Read the model definition and answer for the solid it produces. Units are mm, in the model's axes. Face numbers are marked on the shaded views. A direction names the side the tool comes from. Round coordinates to 2 decimals unless told otherwise and drop trailing zeros. Loops run counter-clockwise (first coordinate to the right, second up) from the corner with the lowest first, then second, coordinate; pieces in that order, holes last. Notation, with made-up numbers: M 64,86 L 86,86 A23 ccw 86,94 Z; hole C -1,18 d11. An arc over 180 degrees is marked long. Write each question's results on one line, items separated by ' | '.
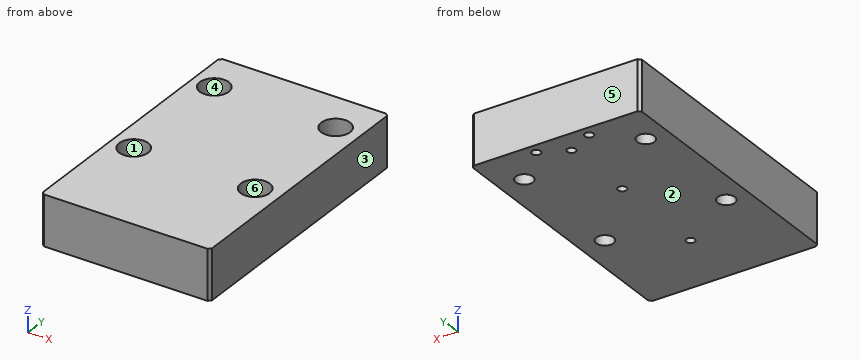
```python
from build123d import *

# Parameters (mm, degrees)
SKETCH_15_W                  = 44
SKETCH_15_H                  = 120
EXTRUDE_1_DEPTH              = 19
HOLE_WIZARD_M4_2_D           = 3.3
HOLE_WIZARD_M4_2_DEPTH       = 11.5
HOLE_WIZARD_M4_2_TIP         = 0.991420021
SKETCH_21_W                  = 44
SKETCH_21_H                  = 18
CUT_EXTRUDE_4_DEPTH          = 19
HOLE_WIZARD_M4_1_D           = 3.3
HOLE_WIZARD_M4_1_DEPTH       = 10.1
HOLE_WIZARD_M4_1_TIP         = 0.991420021
CHAMFER_1_SIZE               = 1
SKETCH_24_W                  = 13.771291576
SKETCH_24_H                  = 102
SKETCH_24_W_2                = 13.032581782
EXTRUDE_2_DEPTH              = 19
HOLE_WIZARD_M6_1_D           = 6.6
HOLE_WIZARD_M6_1_CBORE_D     = 11
HOLE_WIZARD_M6_1_CBORE_DEPTH = 6.4
CHAMFER_2_SIZE               = 1


with BuildPart() as part:
    # 草图15 → 凸台-拉伸1 (new body)
    with BuildSketch(Plane.XY):
        with Locations((3.072247365, -30.72304468)):
            Rectangle(SKETCH_15_W, SKETCH_15_H)
    extrude(amount=EXTRUDE_1_DEPTH)

    # M4 螺纹孔2
    with Locations(Plane(origin=(0, 0, 0), x_dir=(-1, 0, 0), z_dir=(0, 0, -1))):
        with Locations((-3.072247365, 2.27695532), (-3.072247365, -26.72304468), (-3.072247365, -65.72304468)):
            Hole(HOLE_WIZARD_M4_2_D / 2, depth=HOLE_WIZARD_M4_2_DEPTH)
            with Locations((0, 0, -(HOLE_WIZARD_M4_2_DEPTH + HOLE_WIZARD_M4_2_TIP / 2))):  # 118° drill point
                Cone(0, HOLE_WIZARD_M4_2_D / 2, HOLE_WIZARD_M4_2_TIP, mode=Mode.SUBTRACT)

    # 草图21 → 切除-拉伸4 (cut)
    with BuildSketch(Plane.XY.offset(19)):
        with Locations((3.072247365, 20.27695532)):
            Rectangle(SKETCH_21_W, SKETCH_21_H)
    extrude(amount=-CUT_EXTRUDE_4_DEPTH, mode=Mode.SUBTRACT)

    # M4 螺纹孔1
    with Locations(Plane(origin=(0, 0, 0), x_dir=(-1, 0, 0), z_dir=(0, 0, -1))):
        with Locations((-13.072247365, 7.27695532), (6.927752635, 7.27695532)):
            Hole(HOLE_WIZARD_M4_1_D / 2, depth=HOLE_WIZARD_M4_1_DEPTH)
            with Locations((0, 0, -(HOLE_WIZARD_M4_1_DEPTH + HOLE_WIZARD_M4_1_TIP / 2))):  # 118° drill point
                Cone(0, HOLE_WIZARD_M4_1_D / 2, HOLE_WIZARD_M4_1_TIP, mode=Mode.SUBTRACT)

    # 倒角1
    chamfer_1_edges = [part.edges().sort_by_distance(p)[0] for p in [
        (-18.927752635, 11.27695532, 9.5),
        (25.072247365, 11.27695532, 9.5),
        (25.072247365, -90.72304468, 9.5),
        (-18.927752635, -90.72304468, 9.5),
    ]]
    chamfer(chamfer_1_edges, length=CHAMFER_1_SIZE)

    # 草图24 → 凸台-拉伸2 (add)
    with BuildSketch(Plane.XY.offset(19)):
        with Locations((-22.042106847, -39.72304468)):
            Rectangle(SKETCH_24_W, SKETCH_24_H)
        with Locations((28.555956474, -39.72304468)):
            Rectangle(SKETCH_24_W_2, SKETCH_24_H)
    extrude(amount=-EXTRUDE_2_DEPTH)

    # M6 六角凹头螺钉的柱形沉头孔1 (through all)
    with Locations(Plane.XY.offset(19)):
        with Locations((-20.427752635, -4.72304468), (25.572247365, -4.72304468), (25.572247365, -50.70304438), (-20.427752635, -50.72304468)):
            CounterBoreHole(HOLE_WIZARD_M6_1_D / 2, HOLE_WIZARD_M6_1_CBORE_D / 2, HOLE_WIZARD_M6_1_CBORE_DEPTH)

    # 倒角2
    chamfer_2_edges = [part.edges().sort_by_distance(p)[0] for p in [
        (35.072247365, -90.72304468, 9.5),
        (35.072247365, 11.27695532, 9.5),
        (-28.927752635, -90.72304468, 9.5),
        (-28.927752635, 11.27695532, 9.5),
    ]]
    chamfer(chamfer_2_edges, length=CHAMFER_2_SIZE)


solid = part.part
```
1. Find section A-A, the plane x = -22. Give the vertices of the cut face in (y, z), then the cut area to 3 significant figures.
Completed:
outline: M -90.72,0 L -53.62,0 L -53.62,12.6 L -55.99,12.6 L -55.99,19 L -90.72,19 Z; M -47.82,0 L -7.62,0 L -7.62,12.6 L -9.99,12.6 L -9.99,19 L -45.45,19 L -45.45,12.6 L -47.82,12.6 Z; M -1.82,0 L 11.28,0 L 11.28,19 L 0.55,19 L 0.55,12.6 L -1.82,12.6 Z | area: 1,660 mm2
2. Which of the six approach directions +Z, -Z, +X, -X, +Y, -Y give full straight-line access (tool end or side, diameter ignored) to the marked faces 1 and 2?
Completed:
face 1: +Z | face 2: -Z, +X, -X, +Y, -Y
3. Find the intervals of material crossed by L1, parallel to X at y = -4.5, z = 16; L2, parallel to Y at x = -19.5, z = 1.75; L3, parallel to Y at x = 28, z = 4.75, in increasing order.
Completed:
L1: x = -28.93 to -25.92, -14.93 to 20.08, 31.07 to 35.07 | L2: y = -90.72 to -53.89, -47.56 to -7.89, -1.56 to 11.28 | L3: y = -90.72 to -52.94, -48.47 to -6.96, -2.49 to 11.28
4. Given P1, Ø10, axis at x = 25.57, y = -50.7, coming from the +Z side; P2, Ø3, axis at x = 3.07, y = -26.72, coming from the -Z side, each flat-ended and moving along its own axis, determine where each tip first touches the part or whether it passes through.
Completed:
P1: stops at z = 12.6 | P2: stops at z = 11.59
5. Find section B-B, the plane z = 16.75. Give the vertices of the cut face in (x, y), then the cut area to 3 significant figures.
Completed:
outline: M -28.93,-89.72 L -27.93,-90.72 L 34.07,-90.72 L 35.07,-89.72 L 35.07,10.28 L 34.07,11.28 L -27.93,11.28 L -28.93,10.28 Z; hole C -20.43,-50.72 d11; hole C -20.43,-4.72 d11; hole C 25.57,-50.7 d11; hole C 25.57,-4.72 d11 | area: 6,150 mm2
6. Determine the mould class of the marked faces 3, 4, 5 and 6 for opening direction Y: released by +Y, released by -Y, zero draft, split by the parting line, or undercut.
Completed:
face 3: zero draft | face 4: undercut | face 5: released by +Y | face 6: undercut
7. Find section C-C, the plane z = 2.5. Count the separate pieces of the cut face and the enclosed holes in it, then the cut area to 3 significant figures.
Completed:
separate pieces: 1 | enclosed holes: 9 | area: 6,350 mm2
